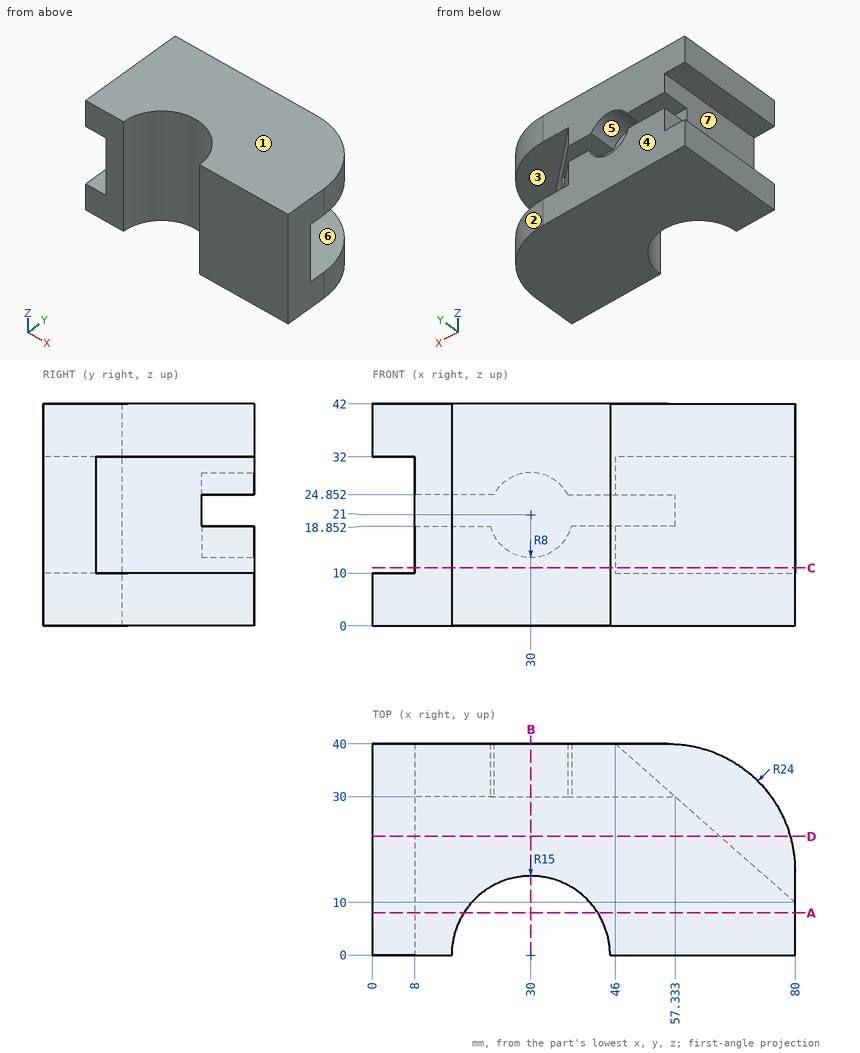
Could you check a few things on this drawing? It's one solid part, dimensions in mm from its lowest x, y, z. A direction names the side the tool comes from. Round coordinates to 2 decimals unless told otherwise and drop trailing zeros. Write each loop counter-clockwise with the first axis right and the second up, starting at its lowest first coordinate (ties: lowest second). Pieces come first, ordered by that corner, then holes.
Q1. If we section it at A-A on y = 8: Write out the boundary of the cut face in (x, z), plus the area to 3 significant figures.
Q2. Which directions (+Z, -Z, +X, -X, +Y, -Y) give clear straight access to the entire face, cutting with the end or side of a thin tool? Please do the marked faces 4, 5, 6 and 7.
Q3. If we section it at C-C on z = 11: Write out the boundary of the cut face in (x, y).
Q4. Will these pins go through, and if not, where does the flat tip stop? P1, Ø1.5, axis at x = 59, z = 12.5, coming from the +Y side; P2, Ø10, axis at y = 16.5, z = 24.5, coming from the -X side; P3, Ø10, axis at y = 29, z = 22, coming from the +X side.
Q5. If we mould it in two halves opening along Z, with no side actions, what happens to the marked faces 1, 2 and 3? For each: +Z half, -Z half, draft (parallel to the pull), parting line (faces both ways), or undercut.
Q6. If we section it at B-B on x = 30: Write out the boundary of the cut face in (y, z).
Q7. Please list where these lines run through material, in increasing order: probe 1 along Z at (x, y) = (20, 37.5); probe 2 along X at (y, z) = (7, 23); probe 3 along X at (y, z) = (10, 40.5).
Q8. If we section it at D-D on y = 22.5: Write out the boundary of the cut face in (x, z), plus the area to 3 significant figures.
Answer below:
1. outline: (0, 0) - (17.31, 0) - (17.31, 42) - (0, 42) - (0, 32) - (8, 32) - (8, 10) - (0, 10) - close; (42.69, 0) - (80, 0) - (80, 42) - (42.69, 42) - close
1. area: 2,120 mm2
2. face 4: +Z, -Z, +X, -X, +Y
2. face 5: +Y
2. face 6: +X, +Y
2. face 7: -X, +Y, -Y
3. outline: (8, 0) - (15, 0) arc R15 cw to (45, 0) - (80, 0) - (80, 10) - (46, 40) - (8, 40) - close
4. P1: stops at y = 29.19
4. P2: stops at x = 8
4. P3: stops at x = 64.13
5. face 1: +Z half
5. face 2: draft
5. face 3: undercut
6. outline: (15, 0) - (40, 0) - (40, 13) - (30, 13) - (30, 29) - (40, 29) - (40, 42) - (15, 42) - close
7. probe 1: z = 0 to 18.85, 24.85 to 42
7. probe 2: x = 8 to 16.73, 43.27 to 80
7. probe 3: x = 0 to 18.82, 41.18 to 80
8. outline: (0, 0) - (79.1, 0) - (79.1, 10) - (65.83, 10) - (65.83, 32) - (79.1, 32) - (79.1, 42) - (0, 42) - (0, 32) - (8, 32) - (8, 10) - (0, 10) - close
8. area: 2,850 mm2
